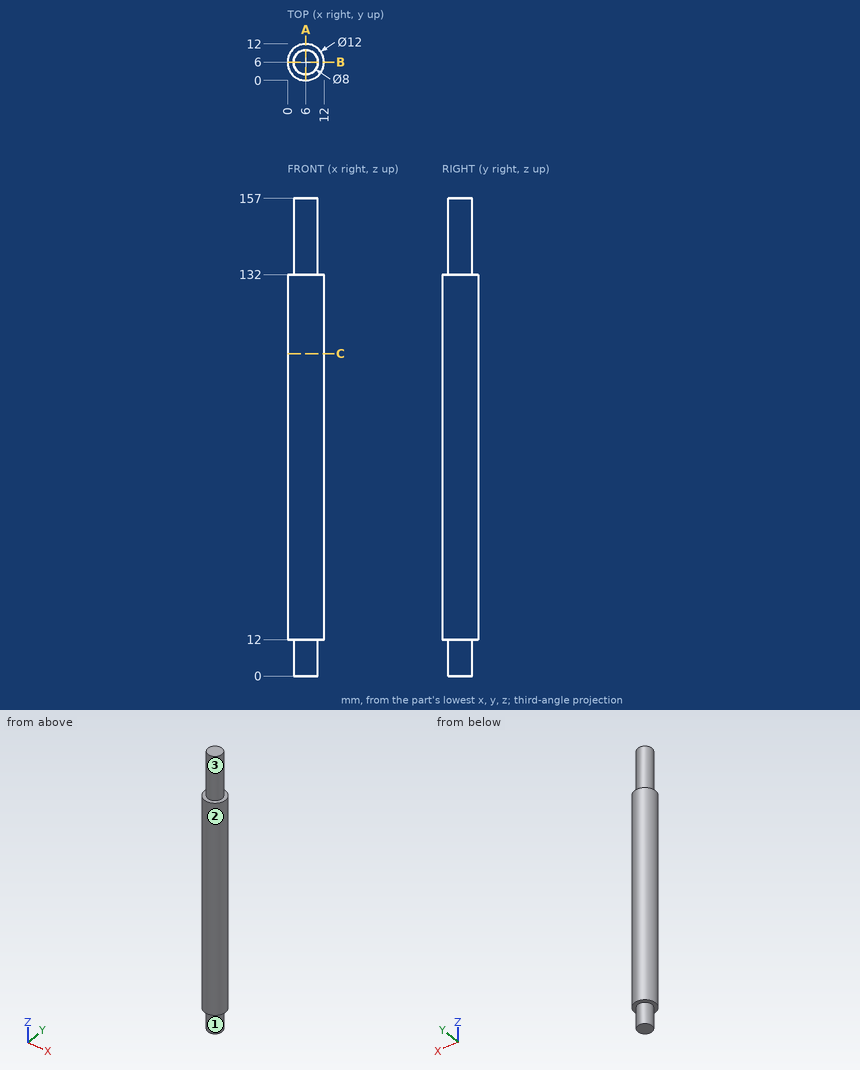
Part print with two shaded views. Sizes in mm from the minimum x, y, z corner. A direction names the side the tool comes from. Round coordinates to 2 decimals unless told otherwise and drop trailing zeros. Order: outer loops, then holes, each group sorted by start corner. A loop starts at its lowest first (then second) coordinate and runs counter-clockwise, first axis right, second up.
(1) Band-saw the part on C-C (z = 106). List the corners of the cut face in (x, y), then the cut area to 3 significant figures.
(2) Band-saw the part on A-A (x = 6). List the corners of the cut face in (y, z).
(3) Drill centre lines: line 1 (Y direction, x = 10.5, z = 44.5); line 2 (Z direction, x = 10.5, y = 9.5); line 3 (Y direction, x = 8.75, z = 107). Where is each one in solid material? Low to high.
(4) 3-axis set-ups, long thin cutter, end or side, ignore diameter. For the marked faces 1, 2 and 3: which of +Z, -Z, +X, -X, +Y, -Y reach the whole face in a straight line?
Verdict:
1. outline: circle Ø12 at (6, 6)
1. area: 113 mm2
2. outline: (0, 12) - (2, 12) - (2, 0) - (10, 0) - (10, 12) - (12, 12) - (12, 132) - (10, 132) - (10, 157) - (2, 157) - (2, 132) - (0, 132) - close
3. line 1: y = 2.03 to 9.97
3. line 2: z = 12 to 132
3. line 3: y = 0.67 to 11.33
4. face 1: -Z
4. face 2: +Z, -Z
4. face 3: +Z
